Geometry: final body of the model. Coordinates: model frame, mm. Face numbers are marked on the shaded views. A direction names the side the tool comes from. Give positions to 0.01 mm unless a question says otherwise; leave off trailing zeros. Write each loop counter-clockwise with the first axis right and the second up, starting at its lowest first coordinate (ties: lowest second). Pieces come first, ordered by that corner, then holes. Notation, with made-up numbers: (-2.5, -4.5) -> (44.5, -4.5) arc R23 cw to (44.5, 20.5) -> close; hole circle Ø3 at (57.5, 13). An arc over 180 degrees is marked (long way). Answer in a Markdown table with one row per item. Add a question column.
Item 1: Material intervals for probe 1 along Y at (x, z) = (0, -16.75); probe 2 along Y at (x, z) = (2, 5); probe 3 along Z at (x, y) = (-7, -43), sorted ascending. Write a range as from..to.
Item 2: First-contact query: P1, Ø5, axis at x = -2, z = -4.5, coming from the +Y side; P2, Ø6, axis at y = -29, z = -9.5, coming from the +X side; P3, Ø13, axis at x = 2.5, z = 1, coming from the -Y side. Flat tips, straight axial feed; report the tip coordinate or a pass-through.
Item 3: Section query A-A on x = 0. State how many separate pieces and enclosed holes the cut face has, plus the area to 3 significant figures.
Item 4: Section query C-C on z = 0. Output: boundary loops of the cut face in (x, y), plus the area to 3 significant figures.
Item 5: Draft query along Y for the marked faces 1, 2 and 3. Return one class per face: +Y half, -Y half, draft (parallel to the pull), parting line (faces both ways), or undercut.
Item 6: Section query D-D on x = -7.5. Output: boundary loops of the cut face in (y, z).
Item 7: Access query for the marked faces 4, 5 and 6. Directions: +Z, -Z, +X, -X, +Y, -Y. A direction counts if a zero-diameter tool reaches every point of the face in a straight line with its end or side. Return the directions, or none.
Item 8: Section query B-B on y = 13. Output: boundary loops of the cut face in (x, z).
```python
from build123d import *

# Parameters (mm, degrees)
SKETCH_1_R               = 5
EXTRUDE_1_DEPTH          = 20
CUT_EXTRUDE_1_DEPTH      = 58.445626465
CUT_EXTRUDE_1_DEPTH_BACK = 58.445626465
SKETCH_2_R               = 16.25
SKETCH_2_W               = 16
SKETCH_2_H               = 60


with BuildPart() as part:
    # 草图1 → 凸台-拉伸1 (new, symmetric)
    with BuildSketch(Plane.XY):
        with BuildLine():
            Line((20, -20), (20, 20))
            Line((20, 20), (9.114378278, 44.114378278))
            ThreePointArc((9.114378278, 44.114378278), (0, 50), (-9.114378278, 44.114378278))
            Line((-9.114378278, 44.114378278), (-20, 20))
            Line((-20, 20), (-20, -20))
            Line((-20, -20), (-9.114378278, -44.114378278))
            ThreePointArc((-9.114378278, -44.114378278), (0, -50), (9.114378278, -44.114378278))
            Line((9.114378278, -44.114378278), (20, -20))
        make_face()
        with Locations((0, 40)):
            Circle(SKETCH_1_R, mode=Mode.SUBTRACT)
        with Locations((10, 0)):
            Circle(SKETCH_1_R, mode=Mode.SUBTRACT)
        with Locations(Location((0, -40, 0), (0, 0, 180))):
            Circle(SKETCH_1_R, mode=Mode.SUBTRACT)
        with Locations(Location((-10, 0, 0), (0, 0, 180))):
            Circle(SKETCH_1_R, mode=Mode.SUBTRACT)
    extrude(amount=EXTRUDE_1_DEPTH, both=True)

    # 草图2 → 切除-拉伸1 (cut, two sides: drawn at the far end of the back side and taken through both)
    with BuildSketch(Plane(origin=(0, 0, 0), x_dir=(0, 0, -1), z_dir=(1, 0, 0)).offset(-CUT_EXTRUDE_1_DEPTH_BACK)):
        Circle(SKETCH_2_R)
        with Locations((0, 50)):
            Rectangle(SKETCH_2_W, SKETCH_2_H)
        with Locations((0, -50)):
            Rectangle(SKETCH_2_W, SKETCH_2_H)
    extrude(amount=CUT_EXTRUDE_1_DEPTH + CUT_EXTRUDE_1_DEPTH_BACK, mode=Mode.SUBTRACT)


solid = part.part
```
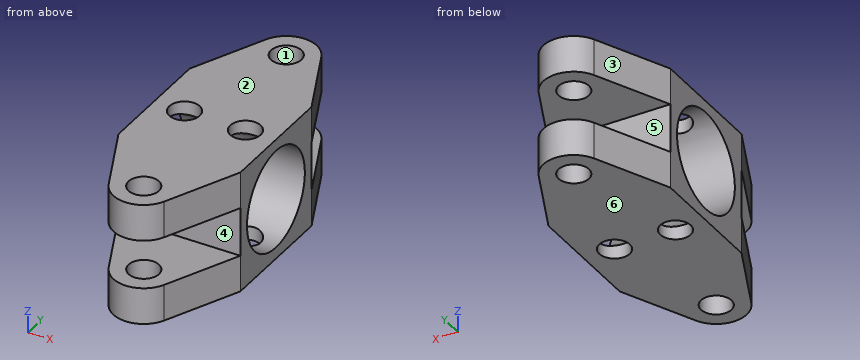
Findings below:
| question | item | result |
|---|---|---|
| 1 | probe 1 | y = -50..-45, -35..35, 45..50 |
| 1 | probe 2 | y = -20..-15.46, 15.46..20 |
| 1 | probe 3 | z = -20..-8, 8..20 |
| 2 | P1 | stops at y = 20 |
| 2 | P2 | stops at x = 17.29 |
| 2 | P3 | stops at y = -20 |
| 3 | separate pieces | 5 |
| 3 | enclosed holes | 1 |
| 3 | area | 1,730 mm^2 |
| 4 | outline | (-20, -20) -> (20, -20) -> (20, -16.25) -> (-20, -16.25) -> close; (-20, 16.25) -> (20, 16.25) -> (20, 20) -> (-20, 20) -> close |
| 4 | area | 300 mm^2 |
| 5 | face 1 | undercut |
| 5 | face 2 | draft |
| 5 | face 3 | +Y half |
| 6 | outline | (-46.61, -20) -> (-4.33, -20) -> (-4.33, -15.66) arc R16.25 cw to (-4.33, 15.66) -> (-4.33, 20) -> (-46.61, 20) -> (-46.61, 8) -> (-20, 8) -> (-20, -8) -> (-46.61, -8) -> close; (4.33, -20) -> (46.61, -20) -> (46.61, -8) -> (20, -8) -> (20, 8) -> (46.61, 8) -> (46.61, 20) -> (4.33, 20) -> (4.33, 15.66) arc R16.25 cw to (4.33, -15.66) -> close |
| 7 | face 4 | +X, -X, -Y |
| 7 | face 5 | +X, -X, +Y |
| 7 | face 6 | -Z, +X, -X, +Y, -Y |
| 8 | outline | (-20, -20) -> (20, -20) -> (20, -9.75) -> (-20, -9.75) -> close; (-20, 9.75) -> (20, 9.75) -> (20, 20) -> (-20, 20) -> close |
